Job drawing, mm, ordinate dimensions from the low corner. One solid piece. A direction names the side the tool comes from. Round coordinates to 2 decimals unless told otherwise and drop trailing zeros. Loops run counter-clockwise (first coordinate to the right, second up) from the corner with the lowest first, then second, coordinate; pieces in that order, holes last. Notation, with made-up numbers: (-20.5, 32.5) - (38.5, 32.5) arc R17 cw to (38.5, 64.5) - close; hole circle Ø3 at (54, -10.75). An arc over 180 degrees is marked (long way). Answer as CSV lines item,"result". Start each with the question number.
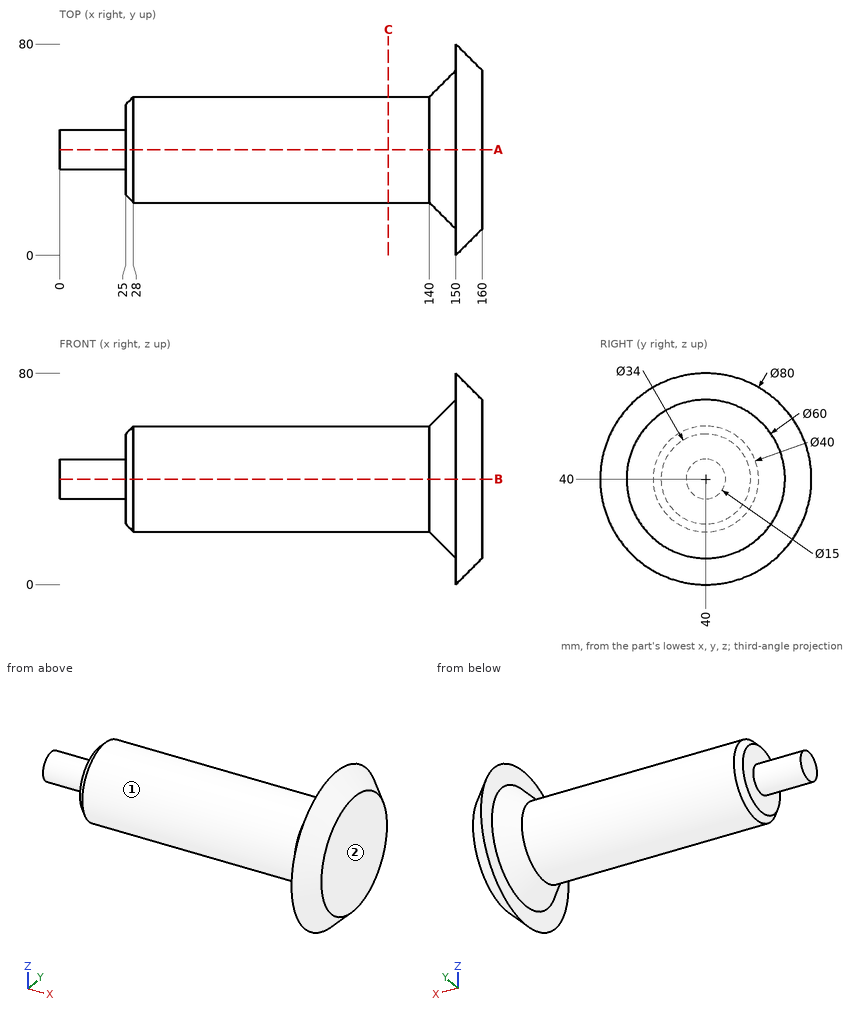
Q1. Pin check, flat tips, straight feed: pin 1 Ø5 at (y, z) = (44.5, 10.5) entering from -X; pin 2 Ø5 at (x, y) = (89.5, 28) entering from +Z; pin 3 Ø10 at (y, z) = (51.5, 43) entering from -X; pin 4 Ø2 at (y, z) = (26.5, 51.5) entering from -X. Stop position of each tip, or through.
Q2. Band-saw the part on C-C, the plane x = 124.5. List the corners of the cut face in (y, z).
Q3. Wall check: probe 1 along X at (y, z) = (34, 51); probe 2 along Z at (x, y) = (65, 40); probe 3 along Y at (x, z) = (58, 38.5). Give the ranges that are in metal, low to high. Write a range as [from, to].
Q4. Band-saw the part on A-A, the plane y = 40. List the corners of the cut face in (x, z).
Q5. Tool access for the marked faces 1 and 2: list every direction of +Z, -Z, +X, -X, +Y, -Y with a clear straight run to the whole face (end or side of a thin tool).
Reported:
1,pin 1,"stops at x = 147.34"
1,pin 2,"stops at z = 57.6"
1,pin 3,"stops at x = 0"
1,pin 4,"stops at x = 25"
2,outline,"circle Ø40 at (40, 40)"
3,probe 1,"x = [25, 160]"
3,probe 2,"z = [20, 60]"
3,probe 3,"y = [20.06, 59.94]"
4,outline,"(0, 32.5) - (25, 32.5) - (25, 23) - (28, 20) - (140, 20) - (150, 10) - (150, 0) - (160, 10) - (160, 70) - (150, 80) - (150, 70) - (140, 60) - (28, 60) - (25, 57) - (25, 47.5) - (0, 47.5) - close"
5,face 1,"-X"
5,face 2,"+Z, -Z, +X, +Y, -Y"
